```python
from build123d import *

# Parameters (mm, degrees)
SKETCH1_R           = 9
BOSS_EXTRUDE1_DEPTH = 40
FILLET1_R           = 10


with BuildPart() as part:
    # Sketch1 → Boss-Extrude1 (new body)
    with BuildSketch(Plane.XY):
        Polygon((70, 0), (70, 50), (145, 50), (145, 0), (700, 0), (700, 100), (0, 100), (0, 0), align=None)
        with Locations((35, 49)):
            Circle(SKETCH1_R, mode=Mode.SUBTRACT)
        with Locations((535, 49)):
            Circle(SKETCH1_R, mode=Mode.SUBTRACT)
    extrude(amount=BOSS_EXTRUDE1_DEPTH)

    # Fillet1
    fillet1_edges = [part.edges().sort_by_distance(p)[0] for p in [
        (145, 0, 20),
        (145, 50, 20),
        (70, 50, 20),
        (70, 0, 20),
        (0, 0, 20),
        (700, 0, 20),
    ]]
    fillet(fillet1_edges, radius=FILLET1_R)


solid = part.part
```
Read the model definition and answer for the solid it produces. Units are mm, in the model's axes. A direction names the side the tool comes from. Give positions to 0.01 mm unless a question says otherwise; leave off trailing zeros. Order: outer loops, then holes, each group sorted by start corner. A loop starts at its lowest first (then second) coordinate and runs counter-clockwise, first axis right, second up. Notation, with made-up numbers: (18, 10) -> (64, 10) arc R4 cw to (64, 14) -> close; hole circle Ø4 at (58, -24). An arc over 180 degrees is marked (long way). One line per item, written item: value. Start each with the question number.
(1) Flat-ended cylindrical pins translate along their axes: P1, Ø11, axis at x = 35, y = 49, coming from the -Z side (3 decimals); P2, Ø20, axis at x = 114, z = 29.5, coming from the -Y side. Find the tip coordinate at first contact, or state that the pin passes through.
(2) For a pull along X with two mould halves and no side action, classify faces 1 (the flat face through (35, 0, 20)), 2 (the flat face through (700, 54, 20)), 3 (the cylindrical face through (543.584, 51.703, 19.72)) as released by +X, released by -X, zero draft, split by the parting line, or undercut.
(3) The part is cut by section B-B (y = 24). Determine the outline of the cut face in (x, z).
(4) A tool of negligible diameter and unlimited length cuts with its end or side. For faces 4 (the flat face through (345, 51, 40)), 5 (the flat face through (107, 50, 20)), from which of +Z, -Z, +X, -X, +Y, -Y can it reach the whole face along a straight path? Write none if from no direction.
(5) Straight lines are drawn through the part: L1, parallel to Y at x = 535, z = 12.5; L2, parallel to X at y = 10, z = 3.5; L3, parallel to X at y = 48, z = 15. For each, find the intervals that lie inside material, in ascending order.
(6) The part is cut by section A-A (x = 35). Determine the outline of the cut face in (y, z), and give its area (3 significant figures).
(7) The part is cut by section C-C (z = 20.5). Determine the outline of the cut face in (x, y).
Taken from the geometry:
1. P1: through
1. P2: y = 50
2. face 1: zero draft
2. face 2: released by +X
2. face 3: undercut
3. outline: (0, 0) -> (70, 0) -> (70, 40) -> (0, 40) -> close; (145, 0) -> (700, 0) -> (700, 40) -> (145, 40) -> close
4. face 4: +Z, +X, -X, +Y, -Y
4. face 5: +Z, -Z, -Y
5. L1: 0 to 40, 58 to 100
5. L2: 0 to 70, 145 to 700
5. L3: 0 to 26.06, 43.94 to 74, 141 to 526.06, 543.94 to 700
6. outline: (0, 0) -> (40, 0) -> (40, 40) -> (0, 40) -> close; (58, 0) -> (100, 0) -> (100, 40) -> (58, 40) -> close
6. area: 3,280 mm^2
7. outline: (0, 10) arc R10 ccw to (10, 0) -> (60, 0) arc R10 ccw to (70, 10) -> (70, 40) arc R10 cw to (80, 50) -> (135, 50) arc R10 cw to (145, 40) -> (145, 10) arc R10 ccw to (155, 0) -> (690, 0) arc R10 ccw to (700, 10) -> (700, 100) -> (0, 100) -> close; hole circle Ø18 at (35, 49); hole circle Ø18 at (535, 49)
